Build history of the part. All positions in model axes, mm. Face numbers are marked on the shaded views. A direction names the side the tool comes from. Round coordinates to 2 decimals unless told otherwise and drop trailing zeros. Write each loop counter-clockwise with the first axis right and the second up, starting at its lowest first coordinate (ties: lowest second). Pieces come first, ordered by that corner, then holes. Notation, with made-up numbers: M 6.5,-8 L 52.5,-8 A18 cw 52.5,21 Z; hole C 79,4.5 d2. An arc over 180 degrees is marked long. Write item = value, one per line.
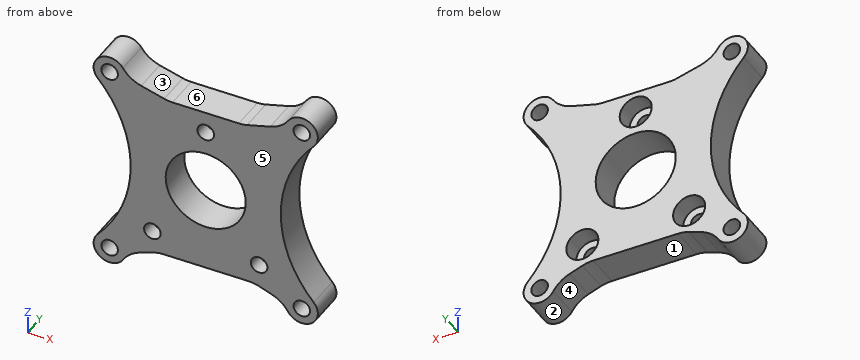
from build123d import *

# Parameters (mm, degrees)
SKETCH_1_R           = 1.55
EXTRUDE_1_DEPTH      = 6.5
FILLET_1_R           = 6
SKETCH_9_R           = 7.5
SKETCH_9_R_2         = 1.55
CUT_EXTRUDE_11_DEPTH = 31.401480227
SKETCH_10_R          = 3
CUT_EXTRUDE_12_DEPTH = 3.5


with BuildPart() as part:
    # 草图1 → 凸台-拉伸1 (new body)
    with BuildSketch(Plane(origin=(0, 0, 0), x_dir=(1, 0, 0), z_dir=(0, 1, 0))):
        with BuildLine():
            Line((-15, 18), (-9, 15.85))
            Line((-9, 15.85), (9, 15.85))
            Line((9, 15.85), (15, 18))
            ThreePointArc((15, 18), (19.079157226, 20.799181966), (20.223613121, 15.986161702))
            ThreePointArc((20.223613121, 15.986161702), (14.060533289, 0), (20.223613121, -15.986161702))
            ThreePointArc((20.223613121, -15.986161702), (19.079157226, -20.799181966), (15, -18))
            Line((15, -18), (7, -15.85))
            Line((7, -15.85), (-7, -15.85))
            Line((-7, -15.85), (-15, -18))
            ThreePointArc((-15, -18), (-19.079157226, -20.799181966), (-20.223613121, -15.986161702))
            ThreePointArc((-20.223613121, -15.986161702), (-14.060533289, 0), (-20.223613121, 15.986161702))
            ThreePointArc((-20.223613121, 15.986161702), (-19.079157226, 20.799181966), (-15, 18))
        make_face()
        with Locations(Location((18, 18, 0), (0, 0, 90))):
            Circle(SKETCH_1_R, mode=Mode.SUBTRACT)
        with Locations(Location((18, -18, 0), (0, 0, 90))):
            Circle(SKETCH_1_R, mode=Mode.SUBTRACT)
        with Locations(Location((-18, -18, 0), (0, 0, 90))):
            Circle(SKETCH_1_R, mode=Mode.SUBTRACT)
        with Locations(Location((-18, 18, 0), (0, 0, 90))):
            Circle(SKETCH_1_R, mode=Mode.SUBTRACT)
    extrude(amount=EXTRUDE_1_DEPTH)

    # 圆角1
    fillet_1_edges = [part.edges().sort_by_distance(p)[0] for p in [
        (15, 3.25, 18),
        (7, 3.25, 15.85),
        (-7, 3.25, 15.85),
        (-15, 3.25, 18),
        (-15, 3.25, -18),
        (-9, 3.25, -15.85),
        (9, 3.25, -15.85),
        (15, 3.25, -18),
    ]]
    fillet(fillet_1_edges, radius=FILLET_1_R)

    # 草图9 → 切除-拉伸11 (cut, through all)
    with BuildSketch(Plane(origin=(0, 6.5, 0), x_dir=(1, 0, 0), z_dir=(0, 1, 0))):
        with Locations(Location((0, 0, 0), (0, 0, 270))):
            Circle(SKETCH_9_R)
        with Locations(Location((10, 11.85, 0), (0, 0, 270))):
            Circle(SKETCH_9_R_2)
        with Locations(Location((0, -11.85, 0), (0, 0, 270))):
            Circle(SKETCH_9_R_2)
        with Locations(Location((-10, 11.85, 0), (0, 0, 270))):
            Circle(SKETCH_9_R_2)
    extrude(amount=-CUT_EXTRUDE_11_DEPTH, mode=Mode.SUBTRACT)

    # 草图10 → 切除-拉伸12 (cut)
    with BuildSketch(Plane(origin=(0, 6.5, 0), x_dir=(1, 0, 0), z_dir=(0, 1, 0))):
        with Locations(Location((-10, 11.85, 0), (0, 0, 270))):
            Circle(SKETCH_10_R)
        with Locations(Location((10, 11.85, 0), (0, 0, 270))):
            Circle(SKETCH_10_R)
        with Locations(Location((0, -11.85, 0), (0, 0, 270))):
            Circle(SKETCH_10_R)
    extrude(amount=-CUT_EXTRUDE_12_DEPTH, mode=Mode.SUBTRACT)


solid = part.part
1. Band-saw the part on A-A (x = 4.5). List the corners of the cut face in (y, z), plus the area to 3 significant figures.
Responses:
outline = M 0,-15.85 L 6.5,-15.85 L 6.5,-6 L 0,-6 Z; M 0,6 L 6.5,6 L 6.5,15.85 L 0,15.85 Z
area = 128 mm²
2. Band-saw the part on D-D (z = -11.85). List the corners of the cut face in (x, y), plus the area to 3 significant figures.
Responses:
outline = M -17.22,0 L -11.55,0 L -11.55,3 L -13,3 L -13,6.5 L -17.22,6.5 Z; M -8.45,0 L 8.45,0 L 8.45,3 L 7,3 L 7,6.5 L -7,6.5 L -7,3 L -8.45,3 Z; M 11.55,0 L 17.22,0 L 17.22,6.5 L 13,6.5 L 13,3 L 11.55,3 Z
area = 163 mm²
3. Flat gauge pins, fed straight in: pin 1 (3 mm diameter, centred on x = 10, z = -12.5, fed in from +Y); pin 2 (1.5 mm diameter, centred on y = 6, z = 0, fed in from -X). Where does each tip first touch, or does it go through?
Responses:
pin_1 = 3
pin_2 = -14.07
4. Band-saw the part on C-C (z = 18). List the corners of the cut face in (x, y).
Responses:
outline = M -21,0 L -19.55,0 L -19.55,6.5 L -21,6.5 Z; M -16.45,0 L -13.83,0 L -13.83,6.5 L -16.45,6.5 Z; M 13.83,0 L 16.45,0 L 16.45,6.5 L 13.83,6.5 Z; M 19.55,0 L 21,0 L 21,6.5 L 19.55,6.5 Z
5. Mould opens along Z. For the marked faces 1, 2 and 3 say: pulls with the +Z half, pulls with the -Z half, needs draft (parallel to the pull), parting line crosses it, or undercut.
Responses:
face_1 = pulls with the -Z half
face_2 = undercut
face_3 = pulls with the +Z half
6. Tool access for the marked faces 4, 5 and 6: list every direction of +Z, -Z, +X, -X, +Y, -Y with a clear straight run to the whole face (end or side of a thin tool).
Responses:
face_4 = -Z, +Y, -Y
face_5 = +Z, -Z, +X, -X, -Y
face_6 = +Z, +Y, -Y
7. Band-saw the part on B-B (y = 3.75). Count the separate pieces of the cut face and the enclosed holes in it, plus the area to 3 significant figures.
Responses:
separate_pieces = 1
enclosed_holes = 8
area = 860 mm²
8. Probe probe 1 along X at (y, z) = (5.55, -11.85); probe 2 along Z at (x, y) = (17, 5.25); probe 3 along X at (y, z) = (4.75, -18.5). List the from-to ranges inside material, lowest first.
Responses:
probe_1 = -17.22 to -13, -7 to 7, 13 to 17.22
probe_2 = -20.83 to -19.18, -16.82 to -11.46, 11.46 to 16.82, 19.18 to 20.83
probe_3 = -20.96 to -19.47, -16.53 to -14.61, 14.61 to 16.53, 19.47 to 20.96
